Check sheet for the modelled part. Datum: model origin and axes. Units: mm. A direction names the side the tool comes from. Coordinates: 2 decimals unless noted, no trailing zeros. Loops run counter-clockwise (first coordinate to the right, second up) from the corner with the lowest first, then second, coordinate; pieces in that order, holes last. Notation, with made-up numbers: M 41,80 L 50,80 A27 ccw 50,108 Z; hole C 88.25,-33 d8. An arc over 180 degrees is marked long. Answer as CSV lines item,"result". Start each with the question number.
from build123d import *

# Parameters (mm, degrees)
SKETCH_1_W               = 1210
SKETCH_1_H               = 240
EXTRUDE_1_DEPTH          = 30
SHELL_1_T                = -2
SKETCH_2_W               = 1210
SKETCH_2_H               = 260
SKETCH_2_W_2             = 1170
SKETCH_2_H_2             = 218
EXTRUDE_2_DEPTH          = 2
CUT_EXTRUDE_1_DEPTH      = 1316
CUT_EXTRUDE_1_DEPTH_BACK = 198
SKETCH_3_R               = 4.5
SKETCH_4_R               = 4.5
CUT_EXTRUDE_2_DEPTH      = 45


with BuildPart() as part:
    # 草图1 → 凸台-拉伸1 (new body)
    with BuildSketch(Plane.XY):
        with Locations((605, 120)):
            Rectangle(SKETCH_1_W, SKETCH_1_H)
    extrude(amount=EXTRUDE_1_DEPTH)

    # 抽壳1
    shell_1_openings = [part.faces().sort_by_distance(p)[0] for p in [
        (605, 120, 30),
    ]]
    offset(amount=SHELL_1_T, openings=shell_1_openings, kind=Kind.INTERSECTION)

    # 草图2 → 凸台-拉伸2 (add)
    with BuildSketch(Plane.XY.offset(30)):
        with Locations((605, 130)):
            Rectangle(SKETCH_2_W, SKETCH_2_H)
        with Locations((605, 129)):
            Rectangle(SKETCH_2_W_2, SKETCH_2_H_2, mode=Mode.SUBTRACT)
    extrude(amount=-EXTRUDE_2_DEPTH)

    # 草图3 → 切除-拉伸1 (cut, two sides: drawn at the far end of the back side and taken through both)
    with BuildSketch(Plane(origin=(2, 0, 0), x_dir=(0, 0, -1), z_dir=(1, 0, 0)).offset(-CUT_EXTRUDE_1_DEPTH_BACK)):
        with Locations(Location((-16, 30, 0), (0, 0, 180))):
            Circle(SKETCH_3_R)
        with Locations(Location((-16, 210, 0), (0, 0, 180))):
            Circle(SKETCH_3_R)
    extrude(amount=CUT_EXTRUDE_1_DEPTH + CUT_EXTRUDE_1_DEPTH_BACK, mode=Mode.SUBTRACT)

    # 草图4 → 切除-拉伸2 (cut)
    with BuildSketch(Plane(origin=(0, 2, 0), x_dir=(1, 0, 0), z_dir=(0, 1, 0))):
        with Locations(Location((30, -16, 0), (0, 0, 270))):
            Circle(SKETCH_4_R)
        with Locations(Location((1180, -16, 0), (0, 0, 270))):
            Circle(SKETCH_4_R)
        with Locations(Location((680, -16, 0), (0, 0, 270))):
            Circle(SKETCH_4_R)
        with Locations(Location((320, -16, 0), (0, 0, 270))):
            Circle(SKETCH_4_R)
        with Locations(Location((740, -16, 0), (0, 0, 270))):
            Circle(SKETCH_4_R)
    extrude(amount=-CUT_EXTRUDE_2_DEPTH, mode=Mode.SUBTRACT)


solid = part.part
Item 1: Sectioned sample at C-C, the plane y = 59.5. Record the boundary of the cut face in (x, z), and give its area (3 significant figures).
Item 2: Set-up check for faces 1 (the face through (513, 15, 30)), 2 (the face through (597, 240, 14)), 3 (the face through (602, 16, 28)): record each of +Z, -Z, +X, -X, +Y, -Y from which the full face is reachable in a straight line by a thin tool's end or side.
Item 3: Sectioned sample at A-A, the plane z = 6.5. Record the boundary of the cut face in (x, y), and give its area (3 significant figures).
Item 4: Material ranges on line 1 (Y direction, x = 0.85, z = 16); line 2 (Y direction, x = 679.5, z = 8.5); line 3 (Z direction, x = 680, y = 0.7), recorded low to high. Write a range as from..to.
Item 5: Go/stop test with flat-tipped pins: pin 1 (4 mm diameter, centred on x = 255.5, y = 93.5, fed in from +Z); pin 2 (14.5 mm diameter, centred on x = 680, z = 16, fed in from +Y); pin 3 (22 mm diameter, centred on x = 836.5, y = 251.5, fed in from -Z). Record where each tip stops, or that it passes through.
Item 6: Sectioned sample at B-B, the plane x = 705. Record the boundary of the cut face in (y, z), and give its area (3 significant figures).
Item 7: Release check for a two-part mould opening along Z. For faces 4 (the face through (2, 118, 15)), 5 (the face through (597, 0, 15)), 6 (the face through (597, 122, 0)) record: released by +Z, released by -Z, zero draft, split by the parting line, or undercut.
Reply:
1,outline,"M 0,0 L 1210,0 L 1210,30 L 1190,30 L 1190,28 L 1208,28 L 1208,2 L 2,2 L 2,28 L 20,28 L 20,30 L 0,30 Z"
1,area,"2,600 mm²"
2,face 1,"+Z, +X, -X, +Y, -Y"
2,face 2,"-Z, +X, -X, +Y"
2,face 3,"none"
3,outline,"M 0,0 L 1210,0 L 1210,240 L 0,240 Z; hole M 2,2 L 1208,2 L 1208,238 L 2,238 Z"
3,area,"5,780 mm²"
4,line 1,"0..25.5, 34.5..205.5, 214.5..240"
4,line 2,"0..2, 238..240"
4,line 3,"0..11.5, 20.5..30"
5,pin 1,"z = 2"
5,pin 2,"y = 240"
5,pin 3,"z = 28"
6,outline,"M 0,0 L 240,0 L 240,28 L 260,28 L 260,30 L 238,30 L 238,2 L 2,2 L 2,28 L 20,28 L 20,30 L 0,30 Z"
6,area,"668 mm²"
7,face 4,"undercut"
7,face 5,"zero draft"
7,face 6,"released by -Z"
